```python
from build123d import *

# Parameters (mm, degrees)
BLOCK_PROFILE_SKETCH_R   = 13
BLOCK_BODY_DEPTH         = 30
TOP_GROOVE_SKETCH_W      = 3
TOP_GROOVE_SKETCH_H      = 14
TOP_GROOVE_CUT_DEPTH     = 91.227490268
SIDE_CROSS_HOLE_SKETCH_R = 7
SIDE_CROSS_HOLE_DEPTH    = 83.152297594


with BuildPart() as part:
    # Block Profile Sketch → Block Body (new body)
    with BuildSketch(Plane.XY):
        Polygon((0, 0), (23, 0), (23, -5), (57, -5), (57, 0), (80, 0), (80, 6), (68, 6), (68, 30), (58, 30), (50, 35), (30, 35), (22, 30), (12, 30), (12, 6), (0, 6), align=None)
        with Locations((40, 16)):
            Circle(BLOCK_PROFILE_SKETCH_R, mode=Mode.SUBTRACT)
    extrude(amount=-BLOCK_BODY_DEPTH)

    # Top Groove Sketch → Top Groove Cut (cut, through all)
    with BuildSketch(Plane(origin=(0, 6, 0), x_dir=(1, 0, 0), z_dir=(0, 1, 0))):
        with Locations((1.5, 15.037121503)):
            Rectangle(TOP_GROOVE_SKETCH_W, TOP_GROOVE_SKETCH_H)
        with Locations((78.5, 15.037121503)):
            Rectangle(TOP_GROOVE_SKETCH_W, TOP_GROOVE_SKETCH_H)
    extrude(amount=-TOP_GROOVE_CUT_DEPTH, mode=Mode.SUBTRACT)

    # Side Cross Hole Sketch → Side Cross Hole (cut, through all)
    with BuildSketch(Plane.ZY.offset(-12)):
        with Locations(Location((-15, 16, 0), (0, 0, 270))):
            Circle(SIDE_CROSS_HOLE_SKETCH_R)
    extrude(amount=-SIDE_CROSS_HOLE_DEPTH, mode=Mode.SUBTRACT)


solid = part.part
```
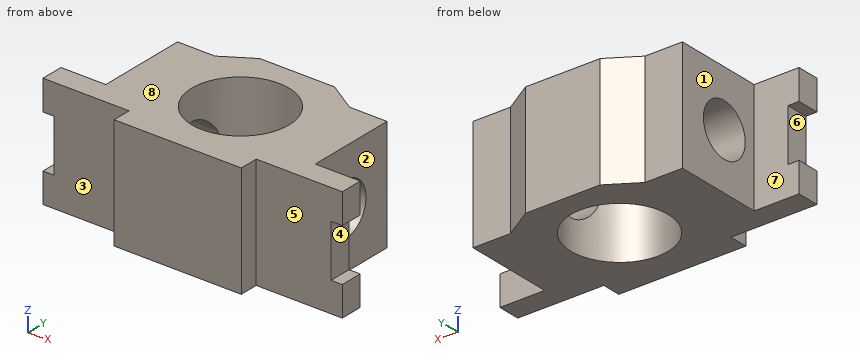
Model file for the job. Use its own axes, mm. Face numbers are marked on the shaded views. A direction names the side the tool comes from. Give positions to 0.01 mm unless a question says otherwise; leave off trailing zeros. Loops run counter-clockwise (first coordinate to the right, second up) from the corner with the lowest first, then second, coordinate; pieces in that order, holes last. Notation, with made-up numbers: (38, 65) -> (82, 65) arc R22 ccw to (82, 75) -> close; hole circle Ø10 at (34.25, 45). An arc over 180 degrees is marked (long way). Use CSV: the item, a comma, the result in double quotes. Start each with the question number.
1) Slice it at B-B on x = 40. Give the cut face in (y, z).
2) Slice it at A-A on y = 16. Give the cut face in (x, z), plus the area to 3 significant figures.
3) Slice it at C-C on z = -2. Give the cut face in (x, y), plus the area to 3 significant figures.
4) Mould opens along Z. For the marked faces 6, 7 and 8 say: released by +Z, released by -Z, zero draft, split by the parting line, or undercut.
5) Tool access for the marked faces 1, 2, 3, 4 and 5: list every direction of +Z, -Z, +X, -X, +Y, -Y with a clear straight run to the whole face (end or side of a thin tool).
6) Wall check: line 1 (Y direction, x = 40, z = -10); line 2 (Y direction, x = 19, z = -15); line 3 (Z direction, x = 59, y = 16). Give the ranges that are in metal, low to high.
7) Flat gauge pins, fed straight in: pin 1 Ø10 at (y, z) = (29, -25.5) entering from -X; pin 2 Ø4 at (y, z) = (-2.5, -16.5) entering from +X; pin 3 Ø13 at (x, z) = (73.5, -21) entering from +Y. Where does each tip first touch, or does it go through?
8) Slice it at D-D on z = -15. Give the cut face in (x, y), plus the area to 3 significant figures.
Computed values:
1,outline,"(-5, -30) -> (3, -30) -> (3, 0) -> (-5, 0) -> close; (29, -30) -> (35, -30) -> (35, 0) -> (29, 0) -> close"
2,outline,"(12, -30) -> (27, -30) -> (27, -22) -> (12, -22) -> close; (12, -8) -> (27, -8) -> (27, 0) -> (12, 0) -> close; (53, -30) -> (68, -30) -> (68, -22) -> (53, -22) -> close; (53, -8) -> (68, -8) -> (68, 0) -> (53, 0) -> close"
2,area,"480 mm^2"
3,outline,"(0, 0) -> (23, 0) -> (23, -5) -> (57, -5) -> (57, 0) -> (80, 0) -> (80, 6) -> (68, 6) -> (68, 30) -> (58, 30) -> (50, 35) -> (30, 35) -> (22, 30) -> (12, 30) -> (12, 6) -> (0, 6) -> close; hole circle Ø26 at (40, 16)"
3,area,"1,600 mm^2"
4,face 6,"undercut"
4,face 7,"zero draft"
4,face 8,"released by +Z"
5,face 1,"+Z, -Z, -X, +Y"
5,face 2,"+Z, -Z, +X, +Y"
5,face 3,"+Z, -Z, -X, -Y"
5,face 4,"+X, +Y, -Y"
5,face 5,"+Z, -Z, +X, -Y"
6,line 1,"y = -5 to 3, 29 to 35"
6,line 2,"y = 0 to 9, 23 to 30"
6,line 3,"z = -30 to -22, -8 to 0"
7,pin 1,"stops at x = 12"
7,pin 2,"stops at x = 57"
7,pin 3,"stops at y = 30"
8,outline,"(3, 0) -> (23, 0) -> (23, -5) -> (57, -5) -> (57, 0) -> (77, 0) -> (77, 6) -> (68, 6) -> (68, 9) -> (50.95, 9) arc R13 cw to (29.05, 9) -> (12, 9) -> (12, 6) -> (3, 6) -> close; (12, 23) -> (29.05, 23) arc R13 cw to (50.95, 23) -> (68, 23) -> (68, 30) -> (58, 30) -> (50, 35) -> (30, 35) -> (22, 30) -> (12, 30) -> close"
8,area,"1,130 mm^2"
